Design review of the part built by this model. Coordinates are the model's own, in mm. A direction names the side the tool comes from. Round coordinates to 2 decimals unless told otherwise and drop trailing zeros. Order: outer loops, then holes, each group sorted by start corner. A loop starts at its lowest first (then second) coordinate and runs counter-clockwise, first axis right, second up. Notation, with made-up numbers: M 11.25,50.25 L 43.25,50.25 A17 cw 43.25,82.25 Z; hole C 22,52.5 d7. An arc over 180 degrees is marked long. Write item = value, one per line. Start each with the question number.
```python
from build123d import *

# Parameters (mm, degrees)
SKETCH1_R                    = 14.5
BOSS_EXTRUDE1_DEPTH          = 20
F_4_5_4_5_DIAMETER_HOLE1_D   = 4.5
SKETCH5_W                    = 34
SKETCH5_H                    = 40
CUT_EXTRUDE1_DEPTH           = 2
M4_TAPPED_HOLE1_D            = 3.3
M4_TAPPED_HOLE1_DEPTH        = 10.1
M4_TAPPED_HOLE1_TIP          = 0.991420021
M5_TAPPED_HOLE1_D            = 4.2
M5_TAPPED_HOLE1_DEPTH        = 14
M5_TAPPED_HOLE1_TIP          = 1.2618073
F_4_0_4_DIAMETER_HOLE1_D     = 4
F_4_0_4_DIAMETER_HOLE1_DEPTH = 12
F_4_0_4_DIAMETER_HOLE1_TIP   = 1.201721238
SKETCH12_W                   = 11
SKETCH12_H                   = 12
CUT_EXTRUDE2_DEPTH           = 121.087468122
M3_TAPPED_HOLE1_D            = 2.5
M3_TAPPED_HOLE1_DEPTH        = 8.5
M3_TAPPED_HOLE1_TIP          = 0.751075774
CHAMFER1_SIZE                = 5
CHAMFER2_SIZE                = 2
SKETCH15_R                   = 4
CUT_EXTRUDE3_DEPTH           = 4.5
FILLET1_R                    = 5
CHAMFER3_SIZE                = 1


with BuildPart() as part:
    # Sketch1 → Boss-Extrude1 (new, symmetric)
    with BuildSketch(Plane.XY):
        Polygon((0, 0), (89, 0), (89, 70), (44, 70), (44, 14), (0, 14), align=None)
        with Locations((69, 38)):
            Circle(SKETCH1_R, mode=Mode.SUBTRACT)
    extrude(amount=BOSS_EXTRUDE1_DEPTH, both=True)

    # Ø4.5 (4.5) Diameter Hole1 (through all)
    with Locations(Plane(origin=(0, 0, 0), x_dir=(-1, 0, 0), z_dir=(0, -1, 0))):
        with Locations((-32, 13), (-6, 13), (-6, -13), (-32, -13)):
            Hole(F_4_5_4_5_DIAMETER_HOLE1_D / 2)

    # Sketch5 → Cut-Extrude1 (cut)
    with BuildSketch(Plane.XZ):
        with Locations((19, 0)):
            Rectangle(SKETCH5_W, SKETCH5_H)
    extrude(amount=-CUT_EXTRUDE1_DEPTH, mode=Mode.SUBTRACT)

    # M4 Tapped Hole1
    with Locations(Plane.XY.offset(20)):
        with Locations((55.564971157, 51.435028843), (82.435028843, 51.435028843), (55.564971157, 24.564971157), (82.435028843, 24.564971157)):
            Hole(M4_TAPPED_HOLE1_D / 2, depth=M4_TAPPED_HOLE1_DEPTH)
            with Locations((0, 0, -(M4_TAPPED_HOLE1_DEPTH + M4_TAPPED_HOLE1_TIP / 2))):  # 118° drill point
                Cone(0, M4_TAPPED_HOLE1_D / 2, M4_TAPPED_HOLE1_TIP, mode=Mode.SUBTRACT)

    # M5 Tapped Hole1
    with Locations(Plane(origin=(0, 70, 0), x_dir=(-1, 0, 0), z_dir=(0, 1, 0))):
        with Locations((-71, -12.5), (-71, 12.5)):
            Hole(M5_TAPPED_HOLE1_D / 2, depth=M5_TAPPED_HOLE1_DEPTH)
            with Locations((0, 0, -(M5_TAPPED_HOLE1_DEPTH + M5_TAPPED_HOLE1_TIP / 2))):  # 118° drill point
                Cone(0, M5_TAPPED_HOLE1_D / 2, M5_TAPPED_HOLE1_TIP, mode=Mode.SUBTRACT)

    # Ø4.0 (4) Diameter Hole1
    with Locations(Plane(origin=(0, 70, 0), x_dir=(-1, 0, 0), z_dir=(0, 1, 0))):
        with Locations((-81, 12.5), (-81, -12.5)):
            Hole(F_4_0_4_DIAMETER_HOLE1_D / 2, depth=F_4_0_4_DIAMETER_HOLE1_DEPTH)
            with Locations((0, 0, -(F_4_0_4_DIAMETER_HOLE1_DEPTH + F_4_0_4_DIAMETER_HOLE1_TIP / 2))):  # 118° drill point
                Cone(0, F_4_0_4_DIAMETER_HOLE1_D / 2, F_4_0_4_DIAMETER_HOLE1_TIP, mode=Mode.SUBTRACT)

    # Sketch12 → Cut-Extrude2 (cut, through all)
    with BuildSketch(Plane.XY.offset(20)):
        with Locations((83.5, 6)):
            Rectangle(SKETCH12_W, SKETCH12_H)
    extrude(amount=-CUT_EXTRUDE2_DEPTH, mode=Mode.SUBTRACT)

    # M3 Tapped Hole1
    with Locations(Plane(origin=(78, 0, 0), x_dir=(0, 0, -1), z_dir=(1, 0, 0))):
        with Locations((-10, 6), (0, 6), (10, 6)):
            Hole(M3_TAPPED_HOLE1_D / 2, depth=M3_TAPPED_HOLE1_DEPTH)
            with Locations((0, 0, -(M3_TAPPED_HOLE1_DEPTH + M3_TAPPED_HOLE1_TIP / 2))):  # 118° drill point
                Cone(0, M3_TAPPED_HOLE1_D / 2, M3_TAPPED_HOLE1_TIP, mode=Mode.SUBTRACT)

    # Chamfer1
    chamfer1_edges = [part.edges().sort_by_distance(p)[0] for p in [
        (89, 70, 0),
    ]]
    chamfer(chamfer1_edges, length=CHAMFER1_SIZE)

    # Chamfer2
    chamfer2_edges = [part.edges().sort_by_distance(p)[0] for p in [
        (44, 70, 0),
        (89, 12, 0),
        (78, 0, 0),
    ]]
    chamfer(chamfer2_edges, length=CHAMFER2_SIZE)

    # Sketch15 → Cut-Extrude3 (cut)
    with BuildSketch(Plane(origin=(0, 14, 0), x_dir=(1, 0, 0), z_dir=(0, 1, 0))):
        with Locations(Location((6, 13, 0), (0, 0, 180))):
            Circle(SKETCH15_R)
        with Locations(Location((32, 13, 0), (0, 0, 180))):
            Circle(SKETCH15_R)
        with Locations(Location((32, -13, 0), (0, 0, 180))):
            Circle(SKETCH15_R)
        with Locations(Location((6, -13, 0), (0, 0, 180))):
            Circle(SKETCH15_R)
    extrude(amount=-CUT_EXTRUDE3_DEPTH, mode=Mode.SUBTRACT)

    # Fillet1
    fillet1_edges = [part.edges().sort_by_distance(p)[0] for p in [
        (44, 14, 0),
    ]]
    fillet(fillet1_edges, radius=FILLET1_R)

    # Chamfer3
    chamfer3_edges = [part.edges().sort_by_distance(p)[0] for p in [
        (0, 7, 20),
        (0, 7, -20),
    ]]
    chamfer(chamfer3_edges, length=CHAMFER3_SIZE)


solid = part.part
```
(1) Consider section C-C, the plane y = 41.5. Write out the cut boundary in (x, z).
(2) Insertion check: pin 1 (10.5 mm diameter, centred on x = 6, z = 13, fed in from -Y); pin 2 (6.5 mm diameter, centred on x = 31.5, z = 14.5, fed in from +Y); pin 3 (5 mm diameter, centred on x = 6, z = -13, fed in from -Y); pin 4 (1 mm diameter, centred on y = 26, z = 2, fed in from -X). Each pin has a flat end and moves straight along its axis. Give the tip position at first contact, or say it passes through.
(3) For faces 5 (the face through (73.69, 5.24, 9.01)), 6 (the face through (2, 1, 0)), 7 (the face through (44, 44, 0)), 8 (the face through (4, 9.5, 11)), list the 3-axis set-ups (+Z, -Z, +X, -X, +Y, -Y) from which the entire face can be reached by the end or side of a thin tool; tool diameter is ignored.
(4) Consider section D-D, the plane x = 66. Write out the cut boundary in (y, z).
(5) Consider section B-B, the plane z = 4.5. Write out the cut boundary in (x, y).
(6) Consider section A-A, the plane x = 6. Write out the cut boundary in (y, z).
(7) For line 1 along X through (y, z) = (4, 13); line 2 along Z through (x, y) = (6, 12); line 3 along Z through (x, y) = (81, 61), list the stretches that pass through material, from the lowest coordinate up. Write a range as [from, to].
(8) Draft analysis for pull direction Z (two halves, no side actions). For faces 1 (the face through (82.21, 51.26, 9.08)), 2 (the face through (43, 16, 0)), 3 (the face through (4, 9.5, -15)), 4 (the face through (81.35, 57.01, -12.48)), state which applies: pulls with the +Z half, pulls with the -Z half, needs draft (parallel to the pull), parting line crosses it, or undercut.
Completed:
q1.outline = M 44,-20 L 54.93,-20 L 54.93,20 L 44,20 Z; M 83.07,-20 L 89,-20 L 89,20 L 83.07,20 Z
q2.pin_1 = 0
q2.pin_2 = 14
q2.pin_3 = 2
q2.pin_4 = 44
q3.face_5 = +X
q3.face_6 = +Z, -Z, -Y
q3.face_7 = +Z, -Z, -X, +Y
q3.face_8 = +Y
q4.outline = M 0,-20 L 23.81,-20 L 23.81,20 L 0,20 Z; M 52.19,-20 L 70,-20 L 70,20 L 52.19,20 Z
q5.outline = M 0,0 L 2,0 L 2,2 L 36,2 L 36,0 L 76,0 L 78,2 L 78,12 L 87,12 L 89,14 L 89,65 L 84,70 L 46,70 L 44,68 L 44,19 A5 cw 39,14 L 0,14 Z; hole C 69,38 d29
q6.outline = M 2,-20 L 14,-20 L 14,-17 L 9.5,-17 L 9.5,-15.25 L 2,-15.25 Z; M 2,-10.75 L 9.5,-10.75 L 9.5,-9 L 14,-9 L 14,9 L 9.5,9 L 9.5,10.75 L 2,10.75 Z; M 2,15.25 L 9.5,15.25 L 9.5,17 L 14,17 L 14,20 L 2,20 Z
q7.line_1 = [0, 3.75], [8.25, 29.75], [34.25, 78]
q7.line_2 = [-20, -17], [-9, 9], [17, 20]
q7.line_3 = [-20, -14.5], [-10.5, 10.5], [14.5, 20]
q8.face_1 = pulls with the +Z half
q8.face_2 = needs draft
q8.face_3 = undercut
q8.face_4 = undercut
